from build123d import *

# Parameters (mm, degrees)
BOSS_EXTRUDE1_DEPTH   = 310
SHELL1_T              = -2
CUT_EXTRUDE1_DEPTH    = 10
CUT_EXTRUDE2_DEPTH    = 397.026111511
SKETCH4_R             = 3
BOSS_EXTRUDE2_DEPTH   = 2
M3_TAPPED_HOLE1_D     = 2.5
M3_TAPPED_HOLE1_DEPTH = 4
CUT_EXTRUDE3_REACH    = 466.348
SKETCH7_W             = 3.5
SKETCH7_H             = 301


with BuildPart() as part:
    # Sketch1 → Boss-Extrude1 (new body)
    with BuildSketch(Plane.XY):
        Polygon((-174.265144247, 0), (-123.224065222, -123.224065222), (0, -174.265144247), (123.224065222, -123.224065222), (174.265144247, 0), (123.224065222, 123.224065222), (0, 174.265144247), (-123.224065222, 123.224065222), align=None)
    extrude(amount=BOSS_EXTRUDE1_DEPTH)

    # Shell1
    shell1_openings = [part.faces().sort_by_distance(p)[0] for p in [
        (0, 0, 0),
    ]]
    offset(amount=SHELL1_T, openings=shell1_openings, kind=Kind.INTERSECTION)

    # Sketch2 → Cut-Extrude1 (cut)
    with BuildSketch(Plane.XY.offset(310)):
        Polygon((111.743562251, 111.743562251), (0, 158.029261243), (-111.743562251, 111.743562251), (-158.029261243, 0), (-111.743562251, -111.743562251), (0, -158.029261243), (111.743562251, -111.743562251), (158.029261243, 0), align=None)
    extrude(amount=-CUT_EXTRUDE1_DEPTH, mode=Mode.SUBTRACT)

    # Sketch3 → Cut-Extrude2 (cut, through all)
    with BuildSketch(Plane.XY.offset(310)):
        Polygon((70.138181093, 169.328548035), (-63.801020235, -154.029288344), (130.028007017, -234.315900213), (263.967208344, 89.041936166), align=None)
    extrude(amount=-CUT_EXTRUDE2_DEPTH, mode=Mode.SUBTRACT)

    # Sketch4 → Boss-Extrude2 (add)
    with BuildSketch(Plane(origin=(60.846665746, 146.896845669, 0), x_dir=(0.9238795325112958, -0.38268343236506785, 0), z_dir=(-0.38268343236506785, -0.9238795325112958, 0))):
        with Locations((-23.217589358, 273.25)):
            Circle(SKETCH4_R)
        with Locations((-10.217589358, 273.25)):
            Circle(SKETCH4_R)
        with Locations((-10.217589358, 26.75)):
            Circle(SKETCH4_R)
        with Locations((-23.217589358, 26.75)):
            Circle(SKETCH4_R)
    extrude(amount=BOSS_EXTRUDE2_DEPTH)

    # M3 Tapped Hole1
    with Locations(Plane(origin=(61.612032611, 148.744604734, 0), x_dir=(0.9238795325112958, -0.38268343236506785, 0), z_dir=(0.38268343236506785, 0.9238795325112958, 0))):
        with Locations((-23.217589358, -26.75), (-10.217589358, -26.75), (-23.217589358, -273.25), (-10.217589358, -273.25)):
            Hole(M3_TAPPED_HOLE1_D / 2, depth=M3_TAPPED_HOLE1_DEPTH)

    # Sketch7 → Cut-Extrude3 (cut, up to next)
    with BuildSketch(Plane(origin=(-61.612032611, -148.744604734, 0), x_dir=(0.9238795325112957, -0.38268343236506797, 0), z_dir=(-0.38268343236506797, -0.9238795325112957, 0)), mode=Mode.PRIVATE) as cut_extrude3_sk1:
        with Locations((-1.75, 150.5)):
            Rectangle(SKETCH7_W, SKETCH7_H)
    cut_extrude3_tool1 = extrude(cut_extrude3_sk1.sketch, amount=-CUT_EXTRUDE3_REACH, mode=Mode.PRIVATE) & part.part
    add(cut_extrude3_tool1.solids().sort_by_distance((-63.228822, -148.074909, 150.5))[0], mode=Mode.SUBTRACT)


solid = part.part
The model under review builds one solid part; all positions refer to its coordinate system, in mm. A direction names the side the tool comes from. Coordinates: 2 decimals unless noted, no trailing zeros. Write each loop counter-clockwise with the first axis right and the second up, starting at its lowest first coordinate (ties: lowest second). Pieces come first, ordered by that corner, then holes. Notation, with made-up numbers: M 21.25,-39 L 49.25,-39 A27 cw 49.25,-17 Z; hole C -25,-38.75 d2. An arc over 180 degrees is marked long. Put each result on its own line as item: value.
1) Wall thickness on probe 1 along Y at (x, z) = (-164, 64); probe 2 along Y at (x, z) = (-89.5, 79); probe 3 along X at (y, z) = (144, 249.5): over which ranges is each line inside the solid? List them lowest first. Write a range as [from, to].
Computed:
probe 1: y = [-24.78, -19.56], [19.56, 24.78]
probe 2: y = [-137.19, -135.03], [135.03, 137.19]
probe 3: x = [-73.07, -67.84]
2) Clearance check with flat-ended pins moving along their axes: pin 1 Ø4 at (y, z) = (-83, 118.5) entering from -X; pin 2 Ø12 at (y, z) = (97.5, 254) entering from +X; pin 3 Ø5 at (x, z) = (-79, 201) entering from -Y; pin 4 Ø10 at (x, y) = (-116, 99) entering from +Z. State where each tip first meets the part, or that it passes through.
Computed:
pin 1: stops at x = -140.71
pin 2: stops at x = -129.23
pin 3: stops at y = -142.58
pin 4: stops at z = 310
3) Add section C-C on y = -40. Give the boundary of the cut face in (x, z), then the cut area to 3 significant figures.
Computed:
outline: M -157.7,0 L -155.53,0 L -155.53,308 L -141.46,308 L -141.46,310 L -157.7,310 Z
area: 699 mm2
4) Add section D-D on x = -69.5. Give the boundary of the cut face in (y, z), then the cut area to 3 significant figures.
Computed:
outline: M -145.48,0 L -143.31,0 L -143.31,308 L -129.24,308 L -129.24,310 L -145.48,310 Z; M 129.24,308 L 143.31,308 L 143.31,0 L 145.48,0 L 145.48,310 L 129.24,310 Z
area: 1,400 mm2
5) Add section A-A on x = -151.5. Give the boundary of the cut face in (y, z).
Computed:
outline: M -54.96,0 L -49.73,0 L -49.73,308 L -15.76,308 L -15.76,310 L -54.96,310 Z; M 15.76,308 L 49.73,308 L 49.73,0 L 54.96,0 L 54.96,310 L 15.76,310 Z
6) Add section B-B on z = 281.5. Give the boundary of the cut face in (x, y).
Computed:
outline: M -174.27,0 L -123.22,-123.22 L -64.85,-147.41 L -64.08,-145.56 L -121.69,-121.69 L -172.1,0 L -121.69,121.69 L 0,172.1 L 60.85,146.9 L 61.61,148.74 L 0,174.27 L -123.22,123.22 Z
7) For faces 4 (the flat face through (-84.199, -123.153, 309.014)), 5 (the flat face through (28.327, 146.296, 309.014)), 6 (the flat face through (-91.696, -134.119, 151.844)), list the 3-axis set-ups (+Z, -Z, +X, -X, +Y, -Y) from which the entire face can be reached by the end or side of a thin tool; tool diameter is ignored.
Computed:
face 4: +Z, -Z, +X
face 5: +Z, -Z, -Y
face 6: -Z, +X
8) Draft analysis for pull direction Y (two halves, no side actions). For faces 1 (the flat face through (-55.09, 135.21, 309.01)), 2 (the flat face through (61.307, 148.007, 155.723)), 3 (the flat face through (-136, 61, 310)), state which applies: released by +Y, released by -Y, zero draft, split by the parting line, or undercut.
Computed:
face 1: undercut
face 2: released by -Y
face 3: zero draft
